```python
from build123d import *
from build123d.topology import SkipClean

# Parameters (mm, degrees)
BASE_ANGLE_PLATE_DEPTH           = 41
FORK_LUG_SKETCH_W                = 140
FORK_LUG_SKETCH_H                = 10
FORK_LUGS_DEPTH                  = 15
LUG_END_FILLET_R15_R             = 15
LUG_PIN_HOLE_SKETCH_R            = 6.045758047
LUG_PIN_HOLE_15_DEPTH            = 80
BASE_MOUNTING_HOLES_SKETCH_R     = 5.5
BASE_MOUNTING_HOLES_SKETCH_R_2   = 5.499920343
BASE_MOUNTING_HOLES_11_DEPTH     = 80
LUG_WEB_DEPTH                    = 10
ARM_PLATE_10MM_DEPTH             = 10
ARM_EXTENSION_40MM_DEPTH         = 40
UPRIGHT_BOSS_BLOCK_SKETCH_W      = 40
UPRIGHT_BOSS_BLOCK_SKETCH_H      = 45
UPRIGHT_BOSS_BLOCK_DEPTH         = 40
BEARING_BOSS_CLEARANCE_CUT_DEPTH = 40
BEARING_BOSS_DEPTH               = 40
BOSS_SLOT_SKETCH_W               = 97.132688683
BOSS_SLOT_SKETCH_H               = 20
BOSS_SLOT_CUT_20MM_DEPTH         = 20


with BuildPart() as part:
    # Base Angle Profile Sketch → Base Angle Plate (new, symmetric)
    with BuildSketch(Plane.XY):
        Polygon((0, 0), (150, 0), (150, 45), (140, 45), (140, 10), (0, 10), align=None)
    extrude(amount=BASE_ANGLE_PLATE_DEPTH, both=True)

    # Fork Lug Sketch → Fork Lugs (add)
    with BuildSketch(Plane(origin=(0, 10, 0), x_dir=(1, 0, 0), z_dir=(0, 1, 0))):
        with Locations((70, 15)):
            Rectangle(FORK_LUG_SKETCH_W, FORK_LUG_SKETCH_H)
        with Locations((70, -15)):
            Rectangle(FORK_LUG_SKETCH_W, FORK_LUG_SKETCH_H)
    extrude(amount=FORK_LUGS_DEPTH)

    # Lug End Fillet R15
    lug_end_fillet_r15_edges = [part.edges().sort_by_distance(p)[0] for p in [
        (0, 25, -15),
        (0, 25, 15),
    ]]
    fillet(lug_end_fillet_r15_edges, radius=LUG_END_FILLET_R15_R)

    # Lug Pin Hole Sketch → Lug Pin Hole _15 (cut)
    with BuildSketch(Plane.XY.offset(20)):
        with Locations((15, 17.5)):
            Circle(LUG_PIN_HOLE_SKETCH_R)
    extrude(amount=-LUG_PIN_HOLE_15_DEPTH, mode=Mode.SUBTRACT)

    # Base Mounting Holes Sketch → Base Mounting Holes _11 (cut)
    with BuildSketch(Plane(origin=(0, 10, 0), x_dir=(1, 0, 0), z_dir=(0, 1, 0))):
        with Locations(Location((110, -30.5, 0), (0, 0, 270))):
            Circle(BASE_MOUNTING_HOLES_SKETCH_R)
        with Locations(Location((50, -30.5, 0), (0, 0, 270))):
            Circle(BASE_MOUNTING_HOLES_SKETCH_R)
        with Locations(Location((110, 30.788589269, 0), (0, 0, 270))):
            Circle(BASE_MOUNTING_HOLES_SKETCH_R)
        with Locations(Location((50, 30.788589269, 0), (0, 0, 270))):
            Circle(BASE_MOUNTING_HOLES_SKETCH_R_2)
    extrude(amount=-BASE_MOUNTING_HOLES_11_DEPTH, mode=Mode.SUBTRACT)

    # Lug Web Sketch → Lug Web (add)
    with BuildSketch(Plane.XY.offset(20)):
        Polygon((109.382207464, 25), (109.382207464, 45), (15, 25), align=None)
    extrude(amount=-LUG_WEB_DEPTH)

    # Arm Profile Sketch → Arm Plate 10mm (add)
    with BuildSketch(Plane(origin=(0, 0, -20), x_dir=(-1, 0, 0), z_dir=(0, 0, -1))):
        Polygon((-140, 25), (-140, 45.242509992), (-110, 45.242509992), (-15, 25), align=None)
    extrude(amount=-ARM_PLATE_10MM_DEPTH)

    # Sketch17_3 → Arm Extension 40mm (add)
    with BuildSketch(Plane(origin=(0, 0, -20), x_dir=(-1, 0, 0), z_dir=(0, 0, -1))):
        Polygon((-140, 25), (-140, 45.242509992), (-110, 45.242509992), (-15, 25), align=None)
    extrude(amount=-ARM_EXTENSION_40MM_DEPTH)

    # Upright Boss Block Sketch → Upright Boss Block (add)
    with BuildSketch(Plane(origin=(110, 45.242509992, 20), x_dir=(-1, 0, 0), z_dir=(0, 0, -1))):
        with Locations((-20, 22.5)):
            Rectangle(UPRIGHT_BOSS_BLOCK_SKETCH_W, UPRIGHT_BOSS_BLOCK_SKETCH_H)
    extrude(amount=UPRIGHT_BOSS_BLOCK_DEPTH)

    # Bearing Boss Sketch → Bearing Boss Clearance Cut (cut)
    with BuildSketch(Plane.XY.offset(20)):
        with BuildLine():
            Line((137.363208202, 77.68412768), (129.363208202, 77.68412768))
            Line((129.363208202, 77.68412768), (121.363208202, 77.68412768))
            ThreePointArc((121.363208202, 77.68412768), (129.363208202, 69.68412768), (137.363208202, 77.68412768))
        make_face()
        with BuildLine():
            Line((121.363208202, 77.68412768), (129.363208202, 77.68412768))
            Line((129.363208202, 77.68412768), (137.363208202, 77.68412768))
            ThreePointArc((137.363208202, 77.68412768), (129.363208202, 85.68412768), (121.363208202, 77.68412768))
        make_face()
        with BuildLine():
            Line((137.363208202, 77.68412768), (129.363208202, 77.68412768))
            Line((129.363208202, 77.68412768), (121.363208202, 77.68412768))
            ThreePointArc((121.363208202, 77.68412768), (129.363208202, 69.68412768), (137.363208202, 77.68412768))
        make_face()
        with BuildLine():
            Line((121.363208202, 77.68412768), (129.363208202, 77.68412768))
            Line((129.363208202, 77.68412768), (137.363208202, 77.68412768))
            ThreePointArc((137.363208202, 77.68412768), (129.363208202, 85.68412768), (121.363208202, 77.68412768))
        make_face()
        with BuildLine():
            Line((110, 90.242509992), (110, 85.812237431))
            ThreePointArc((110, 85.812237431), (111.130972734, 88.104568642), (112.532075332, 90.242509992))
            Line((112.532075332, 90.242509992), (110, 90.242509992))
        make_face()
        with BuildLine():
            ThreePointArc((146.194341072, 90.242509992), (148.592137613, 86.12499693), (150, 81.572935245))
            Line((150, 81.572935245), (150, 90.242509992))
            Line((150, 90.242509992), (146.194341072, 90.242509992))
        make_face()
    extrude(amount=-BEARING_BOSS_CLEARANCE_CUT_DEPTH, mode=Mode.SUBTRACT)

    # Sketch20_3 → Bearing Boss (add)
    with SkipClean():  # the faces are left unmerged after this step: merging them gives an invalid solid
        with BuildSketch(Plane.XY.offset(20)):
            with BuildLine():
                ThreePointArc((146.194341072, 90.242509992), (129.363208202, 98.68412768), (112.532075332, 90.242509992))
                Line((112.532075332, 90.242509992), (146.194341072, 90.242509992))
            make_face()
        extrude(amount=-BEARING_BOSS_DEPTH)

    # Boss Slot Sketch → Boss Slot Cut 20mm (cut)
    with SkipClean():  # the faces are left unmerged after this step: merging them gives an invalid solid
        with BuildSketch(Plane(origin=(-4.444159319, 20.856856955, 0), x_dir=(0.9780435534944176, 0.20840059373238926, 0), z_dir=(-0.20840059373238926, 0.9780435534944176, 0))):
            with Locations((68.447012488, 0)):
                Rectangle(BOSS_SLOT_SKETCH_W, BOSS_SLOT_SKETCH_H)
        extrude(amount=-BOSS_SLOT_CUT_20MM_DEPTH, mode=Mode.SUBTRACT)


solid = part.part
```
Model file for the job. Use its own axes, mm. A direction names the side the tool comes from. Coordinates: 2 decimals unless noted, no trailing zeros. Loops run counter-clockwise (first coordinate to the right, second up) from the corner with the lowest first, then second, coordinate; pieces in that order, holes last. Notation, with made-up numbers: (57, -34) - (78, -34) arc R29 ccw to (78, -7) - close; hole circle Ø3 at (26.25, -17). An arc over 180 degrees is marked (long way). Answer as a JSON object with one key per item and string values. Group by question number.
(1) Tool access for faces 4 (the face through (112.546, 25.336, -0.14)), 5 (the face through (97, 38, -20)), 6 (the face through (29.72, 7.688, -0.14)): list every direction of +Z, -Z, +X, -X, +Y, -Y with a clear straight run to the whole face (end or side of a thin tool).
(2) Flat gauge pins, fed straight in: pin 1 (5 mm diameter, centred on x = 92, y = 30, fed in from +Z); pin 2 (23 mm diameter, centred on y = 33.5, z = -33.5, fed in from -X); pin 3 (8 mm diameter, centred on x = 65, z = 7.5, fed in from -Y); pin 4 (9 mm diameter, centred on x = 8, z = -4.5, fed in from +Y). Where does each tip first touch, or does it go through?
(3) Cut at C-C (z = -3). Give the cut face in (x, y), then the cut area to 3 significant figures.
(4) Cut at D-D (x = 80). Give the cut face in (y, z).
(5) Cut at B-B (y = 17.5). Give the cut face in (x, z), then the cut area to 3 significant figures.
(6) Probe line 1 along X through (y, z) = (4, 30); line 2 along Y through (x, z) = (14.5, -15); line 3 along Z through (x, y) = (79, 15). List the from-to ranges inside material, lowest first.
(7) Two-plate mould, pull along Z, no slides. Class faces 1 (the face through (110, 65, 0)), 2 (the face through (115.453, 5.07, 29.784)), 3 (the face through (86, 9, -41)): released by +Z, released by -Z, zero draft, split by the parting line, or undercut.
(8) Cut at A-A (z = 30.5). Give the cut face in (x, y).
Geometry says:
{
 "1": {"face 4": "-X", "face 5": "-Z, -X, +Y", "face 6": "+Y"},
 "2": {"pin 1": "stops at z = 20", "pin 2": "stops at x = 140", "pin 3": "stops at y = 0", "pin 4": "stops at y = 10"},
 "3": {"outline": "(0, 0) - (150, 0) - (150, 45) - (140, 45) - (140, 45.24) - (150, 45.24) - (150, 81.57) arc R21 ccw to (110, 85.81) - (110, 45.24) - (114.17, 25.68) - (110.97, 25) - (140, 25) - (140, 10) - (40.57, 10) - (19.17, 5.44) - (18.2, 10) - (0, 10) - close; hole circle Ø16 at (129.36, 77.68)", "area": "4,140 mm^2"},
 "4": {"outline": "(0, -41) - (10, -41) - (10, -20) - (38.85, -20) - (38.85, -10) - (10, -10) - (10, 10) - (38.85, 10) - (38.85, 20) - (10, 20) - (10, 41) - (0, 41) - close"},
 "5": {"outline": "(2.01, -20) - (8.95, -20) - (8.95, -10) - (2.01, -10) - close; (2.01, 10) - (8.95, 10) - (8.95, 20) - (2.01, 20) - close; (21.05, -20) - (140, -20) - (140, -41) - (150, -41) - (150, 41) - (140, 41) - (140, 20) - (21.05, 20) - (21.05, 10) - (140, 10) - (140, -10) - (21.05, -10) - close", "area": "3,340 mm^2"},
 "6": {"line 1": "x = 0 to 44.52, 55.48 to 104.52, 115.48 to 150", "line 2": "y = 0 to 11.47, 23.53 to 24.99", "line 3": "z = -20 to -10, 10 to 20"},
 "7": {"face 1": "zero draft", "face 2": "undercut", "face 3": "released by -Z"},
 "8": {"outline": "(0, 0) - (44.5, 0) - (44.5, 10) - (0, 10) - close; (55.5, 0) - (104.5, 0) - (104.5, 10) - (55.5, 10) - close; (115.5, 0) - (150, 0) - (150, 45) - (140, 45) - (140, 10) - (115.5, 10) - close"}
}
